The listing builds one solid part. Answer for the finished solid, in the listing's coordinates (mm). A direction names the side the tool comes from. Round coordinates to 2 decimals unless told otherwise and drop trailing zeros. Order: outer loops, then holes, each group sorted by start corner. A loop starts at its lowest first (then second) coordinate and runs counter-clockwise, first axis right, second up. Notation, with made-up numbers: (79, 88) - (100, 88) arc R13 ccw to (100, 96) - close; hole circle Ø8 at (60.5, 83). An arc over 180 degrees is marked (long way). Use CSV: the item, a comma, the result in double quotes. Start each with the question number.
Item 1: A flat-ended cylindrical pin translates along its axis: P1, Ø5, axis at x = -10.5, y = -31, coming from the +Z side. Find the tip coordinate at first contact, or state that the pin passes through.
Item 2: Find section A-A, the plane x = 0. Give the vertices of the cut face in (y, z).
Item 3: For faces 1 (the flat face through (9.4, -30, 2)), 2 (the cylindrical face through (12.6, -45, 7)), 3 (the flat face through (0, -50, 5)), determine the directions among +Z, -Z, +X, -X, +Y, -Y from which every point of the face is accessible in a straight line to the end or side of a thin tool.
Item 4: Find section C-C, the plane y = -31.5. Give the vertices of the cut face in (x, z), plus the area to 3 significant figures.
Item 5: Determine the mould class of faces 4 (the cylindrical face through (-12.6, -15, 7)), 5 (the flat face through (0, 1, 0)), 6 (the flat face through (23, 47, 5)) for opening direction X: +X half, -X half, draft (parallel to the pull), parting line (faces both ways), or undercut.
Item 6: Find section B-B, the plane z = 1.5. Give the vertices of the cut face in (x, y), plus the area to 3 significant figures.
Item 7: Find section D-D, the plane x = 8.5. Give the vertices of the cut face in (y, z).
Item 8: Straight lines are drawn through the part: line 1 along X through (y, z) = (-28, 5.25); line 2 along Y through (x, z) = (0, 5.75); line 3 along X through (y, z) = (-43, 4.75). For each, find the intervals that lie inside material, in ascending order. Write a range as [from, to].
```python
from build123d import *

# Parameters (mm, degrees)
SKETCH_1_W          = 50
SKETCH_1_H          = 100
EXTRUDE_1_DEPTH     = 10
CUT_EXTRUDE_1_DEPTH = 10
CUT_EXTRUDE_2_DEPTH = 6
CHAMFER_1_SIZE      = 5
SKETCH_4_R          = 4.25
CUT_EXTRUDE_3_DEPTH = 10


with BuildPart() as part:
    # 草图1 → 凸台-拉伸1 (new body)
    with BuildSketch(Plane.XY):
        Rectangle(SKETCH_1_W, SKETCH_1_H)
    extrude(amount=EXTRUDE_1_DEPTH)

    # 草图2 → 切除-拉伸1 (cut)
    with BuildSketch(Plane.XY.offset(10)):
        with BuildLine():
            Line((-9.4, -20), (-9.4, -40))
            ThreePointArc((-9.4, -40), (-12.5, -43.1), (-15.6, -40))
            Line((-15.6, -40), (-15.6, -20))
            ThreePointArc((-15.6, -20), (-12.5, -16.9), (-9.4, -20))
        make_face()
        with BuildLine():
            Line((9.4, -40), (9.4, -20))
            ThreePointArc((9.4, -20), (12.5, -16.9), (15.6, -20))
            Line((15.6, -20), (15.6, -40))
            ThreePointArc((15.6, -40), (12.5, -43.1), (9.4, -40))
        make_face()
    extrude(amount=-CUT_EXTRUDE_1_DEPTH, mode=Mode.SUBTRACT)

    # 草图3 → 切除-拉伸2 (cut)
    with BuildSketch(Plane.XY.offset(10)):
        with BuildLine():
            Line((-7.5, -20), (-7.5, -40))
            ThreePointArc((-7.5, -40), (-12.5, -45), (-17.5, -40))
            Line((-17.5, -40), (-17.5, -20))
            ThreePointArc((-17.5, -20), (-12.5, -15), (-7.5, -20))
        make_face()
        with BuildLine():
            Line((17.5, -20), (17.5, -40))
            ThreePointArc((17.5, -40), (12.5, -45), (7.5, -40))
            Line((7.5, -40), (7.5, -20))
            ThreePointArc((7.5, -20), (12.5, -15), (17.5, -20))
        make_face()
    extrude(amount=-CUT_EXTRUDE_2_DEPTH, mode=Mode.SUBTRACT)

    # 倒角1
    chamfer_1_edges = [part.edges().sort_by_distance(p)[0] for p in [
        (25, -50, 5),
        (-25, -50, 5),
        (-25, 50, 5),
        (25, 50, 5),
    ]]
    chamfer(chamfer_1_edges, length=CHAMFER_1_SIZE)

    # 草图4 → 切除-拉伸3 (cut)
    with BuildSketch(Plane.XY.offset(10)):
        with Locations((0, 35)):
            Circle(SKETCH_4_R)
    extrude(amount=-CUT_EXTRUDE_3_DEPTH, mode=Mode.SUBTRACT)


solid = part.part
```
Worked out:
1,P1,"stops at z = 4"
2,outline,"(-50, 0) - (30.75, 0) - (30.75, 10) - (-50, 10) - close; (39.25, 0) - (50, 0) - (50, 10) - (39.25, 10) - close"
3,face 1,"+Z, -Z"
3,face 2,"+Z"
3,face 3,"+Z, -Z, +X, -X, -Y"
4,outline,"(-25, 0) - (-15.6, 0) - (-15.6, 4) - (-17.5, 4) - (-17.5, 10) - (-25, 10) - close; (-9.4, 0) - (9.4, 0) - (9.4, 4) - (7.5, 4) - (7.5, 10) - (-7.5, 10) - (-7.5, 4) - (-9.4, 4) - close; (15.6, 0) - (25, 0) - (25, 10) - (17.5, 10) - (17.5, 4) - (15.6, 4) - close"
4,area,"330 mm²"
5,face 4,"undercut"
5,face 5,"draft"
5,face 6,"+X half"
6,outline,"(-25, -45) - (-20, -50) - (20, -50) - (25, -45) - (25, 45) - (20, 50) - (-20, 50) - (-25, 45) - close; hole (-15.6, -40) arc R3.1 ccw to (-9.4, -40) - (-9.4, -20) arc R3.1 ccw to (-15.6, -20) - close; hole circle Ø8.5 at (0, 35); hole (9.4, -40) arc R3.1 ccw to (15.6, -40) - (15.6, -20) arc R3.1 ccw to (9.4, -20) - close"
6,area,"4,580 mm²"
7,outline,"(-50, 0) - (50, 0) - (50, 10) - (-17, 10) - (-17, 4) - (-43, 4) - (-43, 10) - (-50, 10) - close"
8,line 1,"x = [-25, -17.5], [-7.5, 7.5], [17.5, 25]"
8,line 2,"y = [-50, 30.75], [39.25, 50]"
8,line 3,"x = [-25, -16.5], [-8.5, 8.5], [16.5, 25]"
